```python
from build123d import *

# Parameters (mm, degrees)
SKETCH_1_W          = 28
SKETCH_1_H          = 20
EXTRUDE_1_DEPTH     = 8
SKETCH_2_R          = 1.65
CUT_EXTRUDE_1_DEPTH = 13


with BuildPart() as part:
    # 草图1 → 凸台-拉伸1 (new, symmetric)
    with BuildSketch(Plane.XY):
        Rectangle(SKETCH_1_W, SKETCH_1_H)
    extrude(amount=EXTRUDE_1_DEPTH, both=True)

    # 草图2 → 切除-拉伸1 (cut, symmetric)
    with BuildSketch(Plane(origin=(0, 0, 0), x_dir=(1, 0, 0), z_dir=(0, 1, 0))):
        with Locations(Location((-8, 0, 0), (0, 0, 270))):
            Circle(SKETCH_2_R)
        with Locations(Location((8, 0, 0), (0, 0, 270))):
            Circle(SKETCH_2_R)
    extrude(amount=CUT_EXTRUDE_1_DEPTH, both=True, mode=Mode.SUBTRACT)


solid = part.part
```
The model under review builds one solid part; all positions refer to its coordinate system, in mm. Coordinates: 2 decimals unless noted, no trailing zeros. Write each loop counter-clockwise with the first axis right and the second up, starting at its lowest first coordinate (ties: lowest second). Pieces come first, ordered by that corner, then holes. Notation, with made-up numbers: (60.5, 6.25) - (84.5, 6.25) arc R17 ccw to (84.5, 31.25) - close; hole circle Ø11 at (-6, -15.75). An arc over 180 degrees is marked (long way). Answer in a Markdown table with one row per item. Add a question column.
Q1. Draft analysis for pull direction X (two halves, no side actions). For faces 1 (the face through (-6.885, 0.14, -1.216)), 2 (the face through (0, 10, 0)), 3 (the face through (14, 0, 0)), state which applies: +X half, -X half, draft (parallel to the pull), parting line (faces both ways), or undercut.
Q2. Consider section A-A on x = 8. Give the boundary of the cut face in (y, z), then the cut area to 3 significant figures.
Q3. Consider section C-C on y = 0.25. Give the boundary of the cut face in (x, z).
Q4. Consider section B-B on z = 0. Give the boundary of the cut face in (x, y).
Q5. To check wall thickness, follow line 1 along X through (y, z) = (5.75, 0); line 2 along X through (y, z) = (5.75, 0.75); line 3 along Z through (x, y) = (-8, -4). State the ranges of each line that lie inside material, in increasing order. Write a range as from..to.
Answers below:
| question | item | result |
|---|---|---|
| 1 | face 1 | undercut |
| 1 | face 2 | draft |
| 1 | face 3 | +X half |
| 2 | outline | (-10, -8) - (10, -8) - (10, -1.65) - (-10, -1.65) - close; (-10, 1.65) - (10, 1.65) - (10, 8) - (-10, 8) - close |
| 2 | area | 254 mm² |
| 3 | outline | (-14, -8) - (14, -8) - (14, 8) - (-14, 8) - close; hole circle Ø3.3 at (-8, 0); hole circle Ø3.3 at (8, 0) |
| 4 | outline | (-14, -10) - (-9.65, -10) - (-9.65, 10) - (-14, 10) - close; (-6.35, -10) - (6.35, -10) - (6.35, 10) - (-6.35, 10) - close; (9.65, -10) - (14, -10) - (14, 10) - (9.65, 10) - close |
| 5 | line 1 | -14..-9.65, -6.35..6.35, 9.65..14 |
| 5 | line 2 | -14..-9.47, -6.53..6.53, 9.47..14 |
| 5 | line 3 | -8..-1.65, 1.65..8 |
